```python
from build123d import *

# Parameters (mm, degrees)
EXTRUDE_1_DEPTH        = 9.5
SKETCH_3_R             = 11
EXTRUDE_2_DEPTH        = 4
SKETCH_4_R             = 11
CUT_EXTRUDE_1_DEPTH    = 4
CUT_EXTRUDE_2_DEPTH    = 4
HOLE_WIZARD_1_D        = 7.3
HOLE_WIZARD_1_DEPTH    = 4.4
PATTERN_LINEAR_1_COUNT = 2
PATTERN_LINEAR_1_PITCH = 8
CUT_EXTRUDE_3_DEPTH    = 2
PATTERN_LINEAR_2_COUNT = 2
PATTERN_LINEAR_2_PITCH = 8


with BuildPart() as part:
    # 草图1 → 凸台-拉伸1 (new body)
    with BuildSketch(Plane.XY):
        Polygon((-14, 3), (-11, 0), (-3, 0), (0, 3), (0, 29), (-11, 29), (-11, 13), (-14, 10), align=None)
    extrude(amount=EXTRUDE_1_DEPTH)

    # 草图3 → 凸台-拉伸2 (add)
    with BuildSketch(Plane.XY.offset(9.5)):
        with Locations(Location((-7, 7, 0), (0, 0, 111.323686263))):
            Circle(SKETCH_3_R)
    extrude(amount=EXTRUDE_2_DEPTH)

    # 草图4 → 切除-拉伸1 (cut)
    with BuildSketch(Plane.XY.offset(9.5)):
        with Locations((-7, 7)):
            Circle(SKETCH_4_R)
        Polygon((-13.9282, 7), (-10.4641, 1.000002798), (-3.5359, 1.000002798), (-0.0718, 7), (-3.5359, 12.999997202), (-10.4641, 12.999997202), align=None, mode=Mode.SUBTRACT)
    extrude(amount=CUT_EXTRUDE_1_DEPTH, mode=Mode.SUBTRACT)

    # 草图2 → 旋转1 (revolve)
    with BuildSketch(Plane(origin=(-7, 0, 0), x_dir=(0, 0, -1), z_dir=(1, 0, 0)), mode=Mode.PRIVATE) as revolve_1_sk:
        Polygon((-20, 7), (-20, 10.233), (-19.233, 11), (1.233, 11), (2, 10.233), (2, 7), align=None)
    revolve(revolve_1_sk.sketch.rotate(Axis((-7, 7, -2), (0, 0, 1)), 270), axis=Axis((-7, 7, -2), (0, 0, 1)))

    # 草图5 → 切除-拉伸2 (cut)
    with BuildSketch(Plane.XY.offset(20)):
        Polygon((-9, 8.154700538), (-9, 5.845299462), (-7, 4.690598923), (-5, 5.845299462), (-5, 8.154700538), (-7, 9.309401077), align=None)
    extrude(amount=-CUT_EXTRUDE_2_DEPTH, mode=Mode.SUBTRACT)

    # 孔1
    with Locations(Plane(origin=(0, 0, 0), x_dir=(0, 0, -1), z_dir=(1, 0, 0))):
        with Locations((-4.75, 24.5)):
            hole_wizard_1 = Hole(HOLE_WIZARD_1_D / 2, depth=HOLE_WIZARD_1_DEPTH)

    # 阵列(线性)1: 孔1 ×2
    with Locations(*[(0, -i * PATTERN_LINEAR_1_PITCH, 0) for i in range(1, PATTERN_LINEAR_1_COUNT)]):
        add(hole_wizard_1, mode=Mode.SUBTRACT)

    # 草图9 → 旋转2 (revolve)
    with BuildSketch(Plane(origin=(0, 24.5, 0), x_dir=(1, 0, 0), z_dir=(0, 1, 0)), mode=Mode.PRIVATE) as revolve_2_sk:
        Polygon((-0.4, -4.75), (-0.4, -7.85), (-0.8, -8.25), (-4.4, -8.25), (-4.4, -4.75), align=None)
    revolve(revolve_2_sk.sketch.rotate(Axis((-4.4, 24.5, 4.75), (1, 0, 0)), 180), axis=Axis((-4.4, 24.5, 4.75), (1, 0, 0)))

    # 草图10 → 旋转3 (revolve)
    with BuildSketch(Plane(origin=(0, 16.5, 0), x_dir=(1, 0, 0), z_dir=(0, 1, 0)), mode=Mode.PRIVATE) as revolve_3_sk:
        Polygon((-0.4, -4.75), (-0.4, -7.85), (-0.8, -8.25), (-4.4, -8.25), (-4.4, -4.75), align=None)
    revolve(revolve_3_sk.sketch.rotate(Axis((-4.4, 16.5, 4.75), (1, 0, 0)), 180), axis=Axis((-4.4, 16.5, 4.75), (1, 0, 0)))

    # 草图11 → 切除-拉伸3 (cut)
    with BuildSketch(Plane(origin=(-0.4, 0, 0), x_dir=(0, 0, -1), z_dir=(1, 0, 0))):
        Polygon((-6.25, 25.366025404), (-6.25, 23.633974596), (-4.75, 22.767949192), (-3.25, 23.633974596), (-3.25, 25.366025404), (-4.75, 26.232050808), align=None)
    cut_extrude_3 = extrude(amount=-CUT_EXTRUDE_3_DEPTH, mode=Mode.SUBTRACT)

    # 阵列(线性)2: 切除-拉伸3 ×2
    with Locations(*[(0, -i * PATTERN_LINEAR_2_PITCH, 0) for i in range(1, PATTERN_LINEAR_2_COUNT)]):
        add(cut_extrude_3, mode=Mode.SUBTRACT)


solid = part.part
```
Read the model definition and answer for the solid it produces. Units are mm, in the model's axes. A direction names the side the tool comes from. Give positions to 0.01 mm unless a question says otherwise; leave off trailing zeros. Write each loop counter-clockwise with the first axis right and the second up, starting at its lowest first coordinate (ties: lowest second). Pieces come first, ordered by that corner, then holes. Notation, with made-up numbers: (17.5, 0) -> (57.5, 0) arc R21 cw to (57.5, 24) -> close; hole circle Ø9 at (36, 80). An arc over 180 degrees is marked (long way). Answer in a Markdown table with one row per item.
1) Section A-A on z = 17.25 is taken. Give the vertices of the cut face in (x, y), plus the area to 3 significant figures.
Results list:
| item | result |
|---|---|
| outline | circle Ø8 at (-7, 7); hole (-9, 5.85) -> (-7, 4.69) -> (-5, 5.85) -> (-5, 8.15) -> (-7, 9.31) -> (-9, 8.15) -> close |
| area | 36.4 mm^2 |
2) Section D-D on y = 16.5 is taken. Give the vertices of the cut face in (x, z), plus the area to 3 significant figures.
Results list:
| item | result |
|---|---|
| outline | (-11, 0) -> (0, 0) -> (0, 1.1) -> (-4.4, 1.1) -> (-4.4, 1.25) -> (-0.8, 1.25) -> (-0.4, 1.65) -> (-0.4, 3.25) -> (-2.4, 3.25) -> (-2.4, 6.25) -> (-0.4, 6.25) -> (-0.4, 7.85) -> (-0.8, 8.25) -> (-4.4, 8.25) -> (-4.4, 8.4) -> (0, 8.4) -> (0, 9.5) -> (-11, 9.5) -> close |
| area | 94.2 mm^2 |
3) A tool of negligible diameter and unlimited length cuts with its end or side. For faces 4 (the flat face through (-1.828, 3.958, 11.472)), 5 (the flat face through (-5, 7, 18)), 6 (the flat face through (-1.78, 9.96, 11.47)), 7 (the flat face through (-1.4, 15.2, 4)), from which of +Z, -Z, +X, -X, +Y, -Y can it reach the whole face along a straight path? Write none if from no direction.
Results list:
| item | result |
|---|---|
| face 4 | +Z, +X, -Y |
| face 5 | +Z |
| face 6 | +Z, +X, +Y |
| face 7 | +X |
4) Section C-C on z = 12.25 is taken. Give the vertices of the cut face in (x, y), plus the area to 3 significant figures.
Results list:
| item | result |
|---|---|
| outline | (-13.93, 7) -> (-10.46, 1) -> (-3.54, 1) -> (-0.07, 7) -> (-3.54, 13) -> (-10.46, 13) -> close |
| area | 125 mm^2 |
5) Section B-B on x = -2 is taken. Give the vertices of the cut face in (y, z).
Results list:
| item | result |
|---|---|
| outline | (1, 0) -> (29, 0) -> (29, 9.5) -> (10.34, 9.5) -> (10.34, 13.5) -> (3.66, 13.5) -> (3.66, 9.5) -> (1, 9.5) -> close; circle Ø7 at (16.5, 4.75); circle Ø7 at (24.5, 4.75); hole circle Ø7.3 at (16.5, 4.75); hole (14.77, 4.75) -> (15.63, 3.25) -> (17.37, 3.25) -> (18.23, 4.75) -> (17.37, 6.25) -> (15.63, 6.25) -> close; hole circle Ø7.3 at (24.5, 4.75); hole (22.77, 4.75) -> (23.63, 3.25) -> (25.37, 3.25) -> (26.23, 4.75) -> (25.37, 6.25) -> (23.63, 6.25) -> close |
6) Determine the mould class of faces 1 (the flat face through (-6, 15, 0)), 2 (the flat face through (-2, 1, 5)), 3 (the flat face through (-0.4, 23, 4)) for opening direction Y: released by +Y, released by -Y, zero draft, split by the parting line, or undercut.
Results list:
| item | result |
|---|---|
| face 1 | zero draft |
| face 2 | released by -Y |
| face 3 | undercut |
7) Each of these flat-tipped pins is pushed along its axis until it touches: pin 1 Ø10 at (y, z) = (23.5, 1.5) entering from +X; pin 2 Ø5 at (y, z) = (17, 5) entering from +X; pin 3 Ø0.7 at (y, z) = (7, 18.5) entering from +X; pin 4 Ø3 at (x, z) = (-8, 12.5) entering from -Y. Where does it stop, or does it pass through?
Results list:
| item | result |
|---|---|
| pin 1 | x = 0 |
| pin 2 | x = -0.4 |
| pin 3 | x = -3 |
| pin 4 | y = 1 |
8) Straight lines are drawn through the part: line 1 (Z direction, x = -5.75, y = 23.5); line 2 (X direction, y = 14, z = 2); line 3 (Y direction, x = -7, z = 14.5). For each, find the intervals that lie inside material, in ascending order. Write a range as [from, to].
Results list:
| item | result |
|---|---|
| line 1 | [0, 9.5] |
| line 2 | [-11, 0] |
| line 3 | [3, 11] |
